from build123d import *

# Parameters (mm, degrees)
SKETCH_1_R          = 20
EXTRUDE_1_DEPTH     = 43
SKETCH_2_R          = 11
CUT_EXTRUDE_1_DEPTH = 10
CUT_EXTRUDE_START   = -7
SKETCH_3_R          = 11
CUT_EXTRUDE_2_DEPTH = 7
SKETCH_4_R          = 8
CUT_EXTRUDE_3_DEPTH = 46.782092569
CHAMFER_1_SIZE      = 0.5


with BuildPart() as part:
    # 草图1 → 凸台-拉伸1 (new body)
    with BuildSketch(Plane.XY):
        Circle(SKETCH_1_R)
    extrude(amount=EXTRUDE_1_DEPTH)

    # 草图2 → 切除-拉伸1 (cut)
    with BuildSketch(Plane.XY.offset(43)):
        Circle(SKETCH_2_R)
    extrude(amount=-CUT_EXTRUDE_1_DEPTH, mode=Mode.SUBTRACT)

    # 草图3 → 切除-拉伸2 (cut)
    with BuildSketch(Plane(origin=(0, 0, 0), x_dir=(-1, 0, 0), z_dir=(0, 0, -1)).offset(CUT_EXTRUDE_START)):
        with Locations(Location((0, 0, 0), (0, 0, 180))):
            Circle(SKETCH_3_R)
    extrude(amount=CUT_EXTRUDE_2_DEPTH, mode=Mode.SUBTRACT)

    # 草图4 → 切除-拉伸3 (cut, through all)
    with BuildSketch(Plane(origin=(0, 0, 7), x_dir=(-1, 0, 0), z_dir=(0, 0, -1))):
        Circle(SKETCH_4_R)
    extrude(amount=-CUT_EXTRUDE_3_DEPTH, mode=Mode.SUBTRACT)

    # 倒角1
    chamfer_1_edges = [part.edges().sort_by_distance(p)[0] for p in [
        (-20, 0, 0),
        (-20, 0, 43),
    ]]
    chamfer(chamfer_1_edges, length=CHAMFER_1_SIZE)


solid = part.part
Could you check a few things on this model? Use its own coordinates, in mm. A direction names the side the tool comes from. Give positions to 0.01 mm unless a question says otherwise; leave off trailing zeros. Order: outer loops, then holes, each group sorted by start corner. A loop starts at its lowest first (then second) coordinate and runs counter-clockwise, first axis right, second up.
Item 1: If we section it at A-A, the plane x = 0: Write out the boundary of the cut face in (y, z).
Item 2: I need wall thicknesses on line 1 (Y direction, x = 0, z = 36.25); line 2 (Y direction, x = 0, z = 16); line 3 (X direction, y = -3, z = 13.5). Which ranges of each line are inside material? Lowest first, please.
Item 3: For faces 1 (the face through (1.73, -7.81, 19.82)), 2 (the face through (-2, 8, 7)), 3 (the face through (-2.38, -10.74, 38.07)), which set-ups out of +Z, -Z, +X, -X, +Y, -Y let a thin tool reach every point of the face, with its end or its side?
Item 4: If we section it at D-D, the plane z = 25: Write out the boundary of the cut face in (x, y), plus the area to 3 significant figures.
Item 5: I'm going to push flat-ended pins straight in: pin 1 (4 mm diameter, centred on y = -7, z = 37.5, fed in from +X); pin 2 (11 mm diameter, centred on x = 2.5, y = 2, fed in from +Z); pin 3 (1.5 mm diameter, centred on y = -12.5, z = 15.5, fed in from -X). Where does each tip first touch, or does it pass through?
Item 6: If we mould it in two halves opening along Y, with no side actions, what happens to faces 4 (the face through (-4.336, -19.524, 21.206)), 5 (the face through (8, -8, 0)), 6 (the face through (-2.38, 10.74, 3.55))? For each: pulls with the +Y half, pulls with the -Y half, needs draft (parallel to the pull), parting line crosses it, or undercut.
Item 7: If we section it at C-C, the plane z = 5: Write out the boundary of the cut face in (x, y), plus the area to 3 significant figures.
Values:
1. outline: (-20, 0.5) - (-19.5, 0) - (-11, 0) - (-11, 7) - (-8, 7) - (-8, 33) - (-11, 33) - (-11, 43) - (-19.5, 43) - (-20, 42.5) - close; (8, 7) - (11, 7) - (11, 0) - (19.5, 0) - (20, 0.5) - (20, 42.5) - (19.5, 43) - (11, 43) - (11, 33) - (8, 33) - close
2. line 1: y = -20 to -11, 11 to 20
2. line 2: y = -20 to -8, 8 to 20
2. line 3: x = -19.77 to -7.42, 7.42 to 19.77
3. face 1: +Z, -Z
3. face 2: -Z
3. face 3: +Z
4. outline: circle Ø40 at (0, 0); hole circle Ø16 at (0, 0)
4. area: 1,060 mm2
5. pin 1: stops at x = 19.36
5. pin 2: stops at z = 33
5. pin 3: stops at x = -16.18
6. face 4: parting line crosses it
6. face 5: needs draft
6. face 6: undercut
7. outline: circle Ø40 at (0, 0); hole circle Ø22 at (0, 0)
7. area: 877 mm2
